For this review, use the dimensioned drawing (mm, ordinates from the lowest corner) and the shaded views. Coordinates: 2 decimals unless noted, no trailing zeros. Write each loop counter-clockwise with the first axis right and the second up, starting at its lowest first coordinate (ties: lowest second). Pieces come first, ordered by that corner, then holes. Notation, with made-up numbers: M -18.75,-10.5 L -7.75,-10.5 A30 ccw -7.75,13.5 Z; hole C 19.5,60 d6. An arc over 180 degrees is marked long. Return JSON: item names as keys, results as strings. Group by question number.
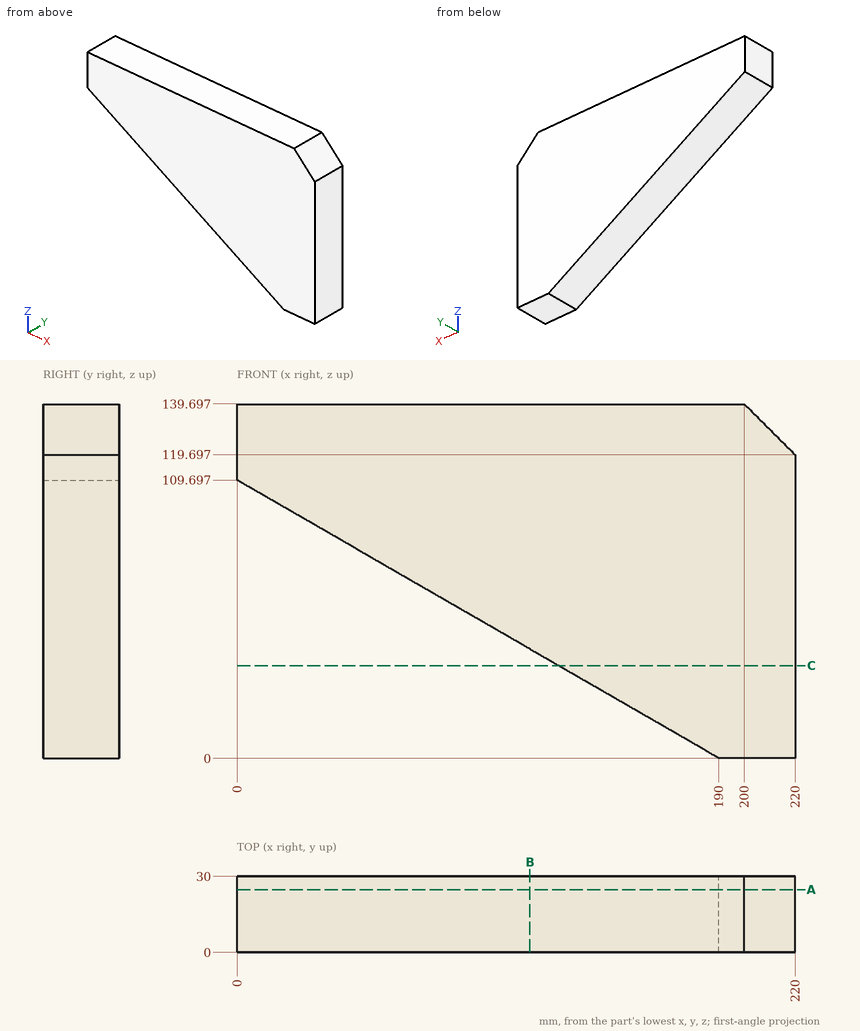
Item 1: Add section A-A (y = 24.75). Write out the cut boundary in (x, z), plus the area to 3 significant figures.
Item 2: For pin 1 (6 mm diameter, centred on x = 175.5, y = 19.5, fed in from -Z); pin 2 (12 mm diameter, centred on y = 5, z = 40, fed in from -X) (1 decimal); pin 3 (12 mm diameter, centred on x = 167, y = 8.5, fed in from -Z) (1 decimal), all flat-tipped, find the tip position at first contact; note any pin that passes through.
Item 3: For line 1 (X direction, y = 5, z = 82.5) (1 decimal); line 2 (X direction, y = 25.5, z = 98); line 3 (Z direction, x = 29, y = 22) (1 decimal), list the stretches that pass through material, from the lowest coordinate up.
Item 4: Add section C-C (z = 36.5). Write out the cut boundary in (x, y), plus the area to 3 significant figures.
Item 5: Add section B-B (x = 115.5). Write out the cut boundary in (y, z).
Geometry check:
{
 "1": {"outline": "M 0,109.7 L 190,0 L 220,0 L 220,119.7 L 200,139.7 L 0,139.7 Z", "area": "20,100 mm^2"},
 "2": {"pin 1": "z = 6.64", "pin 2": "x = 110.3", "pin 3": "z = 9.8"},
 "3": {"line 1": "47.1 to 220", "line 2": "20.26 to 220", "line 3": "93 to 139.7"},
 "4": {"outline": "M 126.78,0 L 220,0 L 220,30 L 126.78,30 Z", "area": "2,800 mm^2"},
 "5": {"outline": "M 0,43.01 L 30,43.01 L 30,139.7 L 0,139.7 Z"}
}
